```python
from build123d import *

# Parameters (mm, degrees)
BOSS_EXTRUDE1_DEPTH = 5


with BuildPart() as part:
    # Sketch1 → Boss-Extrude1 (new, symmetric)
    with BuildSketch(Plane.XY):
        with BuildLine():
            Line((-14.966629547, 10), (-6.6, 10))
            Line((-6.6, 10), (-6.6, 0))
            ThreePointArc((-6.6, 0), (0, -6.6), (6.6, 0))
            Line((6.6, 0), (6.6, 10))
            Line((6.6, 10), (14.966629547, 10))
            ThreePointArc((14.966629547, 10), (0, -18), (-14.966629547, 10))
        make_face()
    extrude(amount=BOSS_EXTRUDE1_DEPTH, both=True)

    # Sketch2 → Cut-Revolve1 (revolve, cut)
    with BuildSketch(Plane.XY, mode=Mode.PRIVATE) as cut_revolve1_sk:
        Polygon((18.861572054, -5.361572054), (18.861572054, -2), (15.5, -2), align=None)
    cut_revolve1 = revolve(cut_revolve1_sk.sketch.rotate(Axis((-24.047626866, -2, 0), (1, 0, 0)), 90), axis=Axis((-24.047626866, -2, 0), (1, 0, 0)), mode=Mode.SUBTRACT)

    # Mirror1: Cut-Revolve1 across plane
    add(cut_revolve1.mirror(Plane(origin=(0, 0, 0), x_dir=(0, 0, 1), z_dir=(1, 0, 0))), mode=Mode.SUBTRACT)


solid = part.part
```
Check sheet for the modelled part. Datum: model origin and axes. Units: mm. A direction names the side the tool comes from. Round coordinates to 2 decimals unless told otherwise and drop trailing zeros. Order: outer loops, then holes, each group sorted by start corner. A loop starts at its lowest first (then second) coordinate and runs counter-clockwise, first axis right, second up.
1) Mould release check, pull along X, two halves, no side actions. Record for faces 1 (the conical face through (-16.212, -1.294, 0.093)), 2 (the flat face through (0, -7, 5)), 3 (the cylindrical face through (-0.1, -6.6, 0.1)): +X half, -X half, draft (parallel to the pull), parting line (faces both ways), or undercut.
2) Scan lines: line 1 (Y direction, x = -10, z = -1.25); line 2 (X direction, y = -6, z = 1.5); line 3 (X direction, y = 1, z = 1.5). Record each from-to range of solid material in increasing order.
3) Section check C-C (x = 0). Record the boundary of the cut face in (y, z).
4) Section check B-B (z = -4.25). Record the boundary of the cut face in (x, y), and give its area (3 significant figures).
5) Tool access check on faces 4 (the flat face through (-6.6, 5, 0)), 5 (the flat face through (-11, 10, 0)). Record the directions out of +Z, -Z, +X, -X, +Y, -Y that give a thin tool (end or side, any length) a straight path to the whole face; none if there is none.
6) Go/stop test with flat-tipped pins: pin 1 Ø2 at (x, z) = (-2.5, 0.5) entering from +Y; pin 2 Ø6 at (x, z) = (-14, -1.5) entering from -Y. Record where each tip stops, or that it passes through.
7) Section check A-A (y = -6). Record the boundary of the cut face in (x, z), and give its area (3 significant figures).
8) Section check D-D (y = -13.5). Record the boundary of the cut face in (x, z), and give its area (3 significant figures).
Result:
1. face 1: -X half
1. face 2: draft
1. face 3: undercut
2. line 1: y = -14.97 to 10
2. line 2: x = -16.97 to -2.75, 2.75 to 16.97
2. line 3: x = -17.97 to -6.6, 6.6 to 17.97
3. outline: (-18, -5) - (-6.6, -5) - (-6.6, 5) - (-18, 5) - close
4. outline: (-14.97, 10) arc R18 ccw (long way) to (14.97, 10) - (6.6, 10) - (6.6, 0) arc R6.6 cw to (-6.6, 0) - (-6.6, 10) - close
4. area: 649 mm2
5. face 4: +Z, -Z, +Y
5. face 5: +Z, -Z, +X, -X, +Y
6. pin 1: stops at y = -5.6
6. pin 2: stops at y = -14.25
7. outline: (-16.97, -5) - (-2.75, -5) - (-2.75, 5) - (-16.97, 5) - close; (2.75, -5) - (16.97, -5) - (16.97, 5) - (2.75, 5) - close
7. area: 284 mm2
8. outline: (-11.91, -5) - (11.91, -5) - (11.91, 5) - (-11.91, 5) - close
8. area: 238 mm2
